Source: CAD feature listing. Evaluate the final solid. Frame: model axes, mm. Coordinates: 2 decimals unless noted, no trailing zeros. Loops run counter-clockwise (first coordinate to the right, second up) from the corner with the lowest first, then second, coordinate; pieces in that order, holes last.
Item 1: Section query A-A, the plane x = 53. Return the cut outline in (y, z), then the cut area to 3 significant figures.
Item 2: Line query: probe 1 along X at (y, z) = (1.15, -38.5); probe 2 along X at (y, z) = (1.6, -37.5). Output: solid intervals per line, ascending.
Item 3: Pin query (flat end, axial travel): pin 1 Ø2.5 at (x, z) = (53, 38.5) entering from -Y. Return the tip coordinate at first contact, or that it passes through.
Item 4: Pull-direction query (X, two-part tool) for faces 1 (the cylindrical face through (53.9, 0.9, -37.3)), 2 (the flat face through (-1, 0, -1)); classes: +X half, -X half, draft (parallel to the pull), parting line (faces both ways), or undercut.
Item 5: Section query B-B, the plane z = -38.5. Return the cut outline in (x, y).
```python
from build123d import *

# Parameters (mm, degrees)
SKETCH_1_W      = 111.5
SKETCH_1_H      = 82.6
SKETCH_1_R      = 1.5
EXTRUDE_1_DEPTH = 1.75


with BuildPart() as part:
    # 草图1 → 凸台-拉伸1 (new body)
    with BuildSketch(Plane(origin=(0, 0, 0), x_dir=(1, 0, 0), z_dir=(0, 1, 0))):
        Rectangle(SKETCH_1_W, SKETCH_1_H)
        with Locations(Location((-53, 38.5, 0), (0, 0, 270))):
            Circle(SKETCH_1_R, mode=Mode.SUBTRACT)
        with Locations(Location((53, 38.5, 0), (0, 0, 90))):
            Circle(SKETCH_1_R, mode=Mode.SUBTRACT)
        with Locations(Location((53, -38.5, 0), (0, 0, 270))):
            Circle(SKETCH_1_R, mode=Mode.SUBTRACT)
        with Locations(Location((-53, -38.5, 0), (0, 0, 90))):
            Circle(SKETCH_1_R, mode=Mode.SUBTRACT)
    extrude(amount=EXTRUDE_1_DEPTH)


solid = part.part
```
Verdict:
1. outline: (0, -41.3) - (1.75, -41.3) - (1.75, -40) - (0, -40) - close; (0, -37) - (1.75, -37) - (1.75, 37) - (0, 37) - close; (0, 40) - (1.75, 40) - (1.75, 41.3) - (0, 41.3) - close
1. area: 134 mm2
2. probe 1: x = -55.75 to -54.5, -51.5 to 51.5, 54.5 to 55.75
2. probe 2: x = -55.75 to -54.12, -51.88 to 51.88, 54.12 to 55.75
3. pin 1: passes through
4. face 1: undercut
4. face 2: draft
5. outline: (-55.75, 0) - (-54.5, 0) - (-54.5, 1.75) - (-55.75, 1.75) - close; (-51.5, 0) - (51.5, 0) - (51.5, 1.75) - (-51.5, 1.75) - close; (54.5, 0) - (55.75, 0) - (55.75, 1.75) - (54.5, 1.75) - close
